Check sheet for the drawn part. Datum: minimum x, y, z corner. Units: mm. A direction names the side the tool comes from. Round coordinates to 2 decimals unless told otherwise and drop trailing zeros. Order: outer loops, then holes, each group sorted by start corner. A loop starts at its lowest first (then second) coordinate and runs counter-clockwise, first axis right, second up. Notation, with made-up numbers: M 49,80 L 69,80 A7 ccw 69,85 Z; hole C 4.25,48.5 d9. An arc over 180 degrees is marked long. Write item = value, one per line. Start each with the question number.
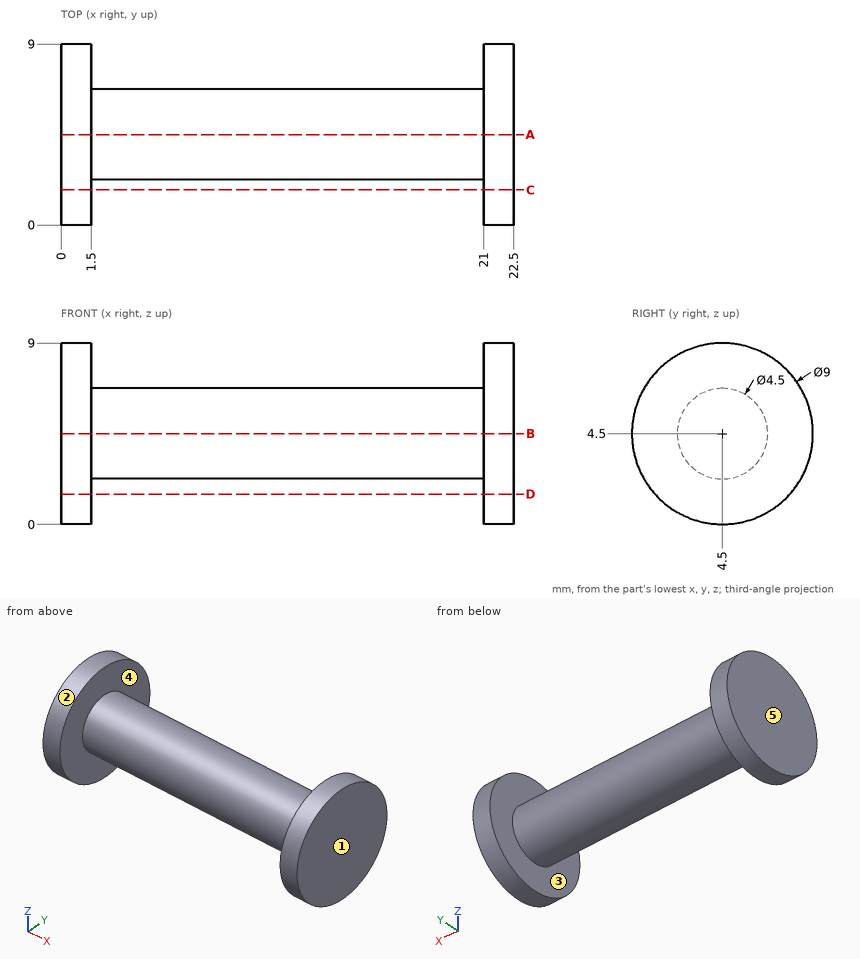
1) Cross-section at C-C, the plane y = 1.75. Enter the section's corners in (x, z).
2) Release check for a two-part mould opening along X. For the marked faces 1, 2 and 3 record: pulls with the +X half, pulls with the -X half, needs draft (parallel to the pull), parting line crosses it, or undercut.
3) Access from +Z, -Z, +X, -X, +Y, -Y to the whole of each face (thin tool, end or side, straight path). Record for the marked faces 4 and 5.
4) Scan lines: probe 1 along X at (y, z) = (0.5, 6.25); probe 2 along Z at (x, y) = (20.75, 4.5); probe 3 along Y at (x, z) = (4.75, 5.5). Record each from-to range of solid material in increasing order.
5) Cross-section at A-A, the plane y = 4.5. Enter the section's corners in (x, z), then the cut area to 3 significant figures.
6) Cross-section at D-D, the plane z = 1.5. Enter the section's corners in (x, y), then the cut area to 3 significant figures.
7) Gauge pin test, flat ends, axial feed: P1, Ø1.5, axis at x = 10.5, z = 4.5, coming from the -Y side; P2, Ø4, axis at x = 5, y = 6, coming from the +Z side. Record the tip position at first contact, or that the pin passes through.
Geometry results:
q1.outline = M 0,0.94 L 1.5,0.94 L 1.5,8.06 L 0,8.06 Z; M 21,0.94 L 22.5,0.94 L 22.5,8.06 L 21,8.06 Z
q2.face_1 = pulls with the +X half
q2.face_2 = needs draft
q2.face_3 = undercut
q3.face_4 = none
q3.face_5 = +Z, -Z, -X, +Y, -Y
q4.probe_1 = 0 to 1.5, 21 to 22.5
q4.probe_2 = 2.25 to 6.75
q4.probe_3 = 2.48 to 6.52
q5.outline = M 0,0 L 1.5,0 L 1.5,2.25 L 21,2.25 L 21,0 L 22.5,0 L 22.5,9 L 21,9 L 21,6.75 L 1.5,6.75 L 1.5,9 L 0,9 Z
q5.area = 115 mm^2
q6.outline = M 0,1.15 L 1.5,1.15 L 1.5,7.85 L 0,7.85 Z; M 21,1.15 L 22.5,1.15 L 22.5,7.85 L 21,7.85 Z
q6.area = 20.1 mm^2
q7.P1 = 2.25
q7.P2 = 6.75
